from build123d import *

# Parameters (mm, degrees)
BLOCK_BODY_DEPTH        = 21
BORE_18_SKETCH_R        = 9
BORE_18_X_40_DEEP_DEPTH = 40


with BuildPart() as part:
    # Block Profile Sketch → Block Body (new, symmetric)
    with BuildSketch(Plane.XY):
        Polygon((30, 0), (-30, 0), (-30, 30), (15, 50), (30, 50), align=None)
    extrude(amount=BLOCK_BODY_DEPTH, both=True)

    # Bore Ø18 Sketch → Bore Ø18 x 40 Deep (cut)
    with BuildSketch(Plane(origin=(30, 0, 0), x_dir=(0, 0, -1), z_dir=(1, 0, 0))):
        with Locations(Location((0, 25, 0), (0, 0, 90))):
            Circle(BORE_18_SKETCH_R)
    extrude(amount=-BORE_18_X_40_DEEP_DEPTH, mode=Mode.SUBTRACT)


solid = part.part
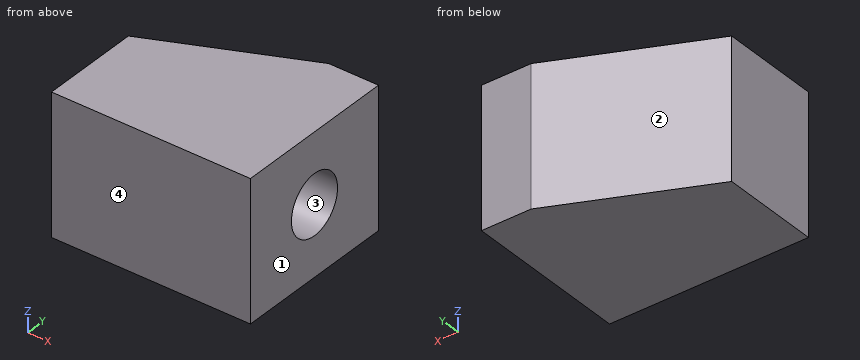
Model file for the job. Use its own axes, mm. Face numbers are marked on the shaded views. Give positions to 0.01 mm unless a question says otherwise; leave off trailing zeros. Loops run counter-clockwise (first coordinate to the right, second up) from the corner with the lowest first, then second, coordinate; pieces in that order, holes last. Notation, with made-up numbers: (-27.5, 53) -> (15.5, 53) arc R10 ccw to (15.5, 62) -> close; hole circle Ø6 at (57.25, 52.25). An arc over 180 degrees is marked (long way). Use a Markdown table: item, result. Add a question column.
(1) Wall check: line 1 along Z through (x, y) = (2, 25); line 2 along Z through (x, y) = (6, 17.5); line 3 along X through (y, z) = (43.5, 12.5) (3 decimals). Give the ranges that are in metal, low to high.
(2) Slice it at A-A on y = 25. List the corners of the cut face in (x, z).
(3) Slice it at D-D on z = 11. List the corners of the cut face in (x, y), and give its area (3 significant figures).
(4) Mould opens along Y. For the marked faces 1, 2, 3 and 4 say: +Y half, -Y half, draft (parallel to the pull), parting line (faces both ways), or undercut.
(5) Slice it at C-C on z = 0. List the corners of the cut face in (x, y), and give its area (3 significant figures).
(6) Slice it at B-B on x = 25.5. List the corners of the cut face in (y, z), and give its area (3 significant figures).
(7) Drop a flat-ended pin along its axis: pin 1 Ø4 at (x, z) = (-20, 5) entering from +Y. Give the stop position or say it passes through.
Filled sheet:
| question | item | result |
|---|---|---|
| 1 | line 1 | -21 to -9, 9 to 21 |
| 1 | line 2 | -21 to -4.97, 4.97 to 21 |
| 1 | line 3 | 0.375 to 30 |
| 2 | outline | (-30, -21) -> (30, -21) -> (30, -9) -> (-10, -9) -> (-10, 9) -> (30, 9) -> (30, 21) -> (-30, 21) -> close |
| 3 | outline | (-30, 0) -> (30, 0) -> (30, 50) -> (15, 50) -> (-30, 30) -> close |
| 3 | area | 2,550 mm2 |
| 4 | face 1 | draft |
| 4 | face 2 | +Y half |
| 4 | face 3 | undercut |
| 4 | face 4 | -Y half |
| 5 | outline | (-30, 0) -> (30, 0) -> (30, 16) -> (-10, 16) -> (-10, 34) -> (30, 34) -> (30, 50) -> (15, 50) -> (-30, 30) -> close |
| 5 | area | 1,830 mm2 |
| 6 | outline | (0, -21) -> (50, -21) -> (50, 21) -> (0, 21) -> close; hole circle Ø18 at (25, 0) |
| 6 | area | 1,850 mm2 |
| 7 | pin 1 | y = 35.33 |
